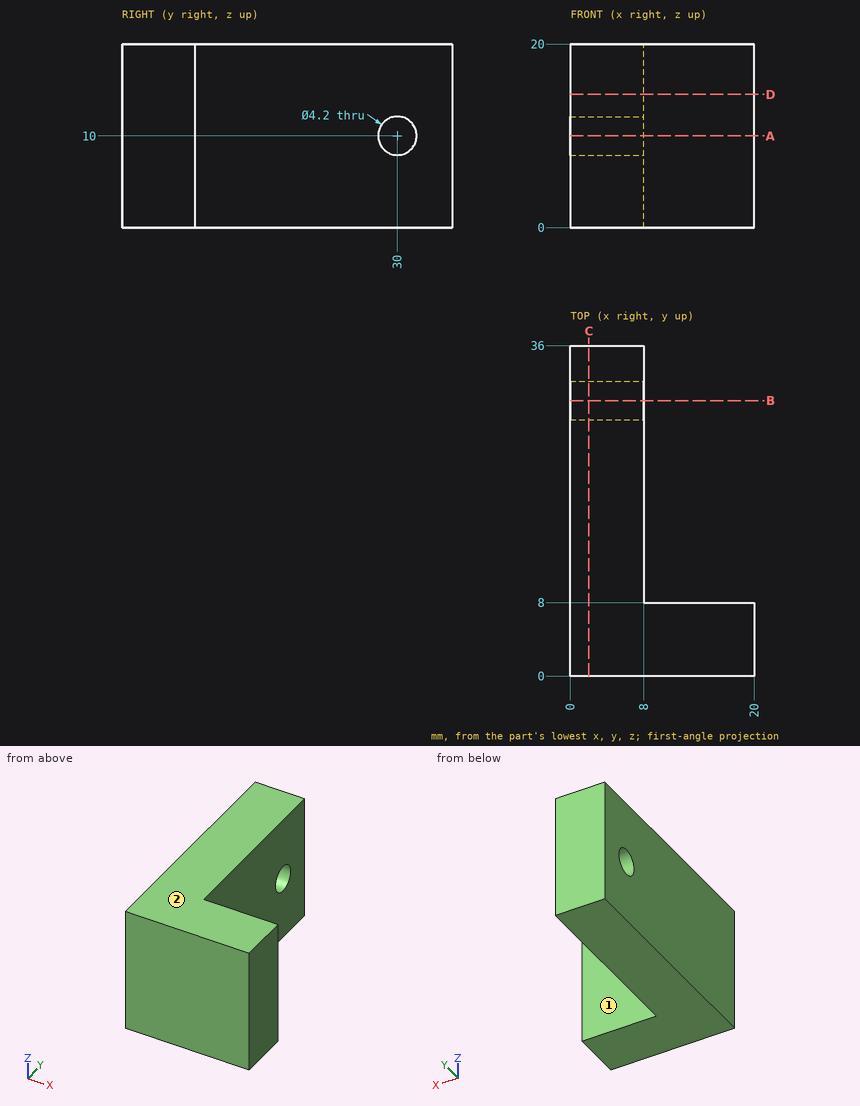
Could you check a few things on this drawing? It's one solid part, dimensions in mm from its lowest x, y, z. A direction names the side the tool comes from. Give positions to 0.01 mm unless a question says otherwise; leave off trailing zeros. Order: outer loops, then holes, each group sorted by start corner. A loop starts at its lowest first (then second) coordinate and runs counter-clockwise, first axis right, second up. Notation, with made-up numbers: (64, 61.5) - (106, 61.5) arc R20 ccw to (106, 78.5) - close; hole circle Ø11 at (21, 19.5). An arc over 180 degrees is marked (long way). Answer as a JSON object with one key per item and string values. Group by question number.
Item 1: Which directions (+Z, -Z, +X, -X, +Y, -Y) give clear straight access to the entire face, cutting with the end or side of a thin tool? Please do the marked faces 1 and 2.
Item 2: For P1, Ø5.5, axis at y = 30, z = 10, coming from the +X side; P2, Ø9.5, axis at x = 14, z = 8.5, coming from the +Y side, each with a flat end and sliding along its axis, tell me the tip position at first contact or that it passes through.
Item 3: If we section it at C-C on x = 2: Please give me the cut outline in (y, z).
Item 4: If we section it at B-B on y = 30: Please give me the cut outline in (x, z).
Item 5: If we section it at A-A on z = 10: Please give me the cut outline in (x, y), and give its area (3 significant figures).
Item 6: If we section it at D-D on z = 14.5: Please give me the cut outline in (x, y).
Item 7: Please list where these lines run through material, in increasing order: probe 1 along Y at (x, z) = (4.25, 10); probe 2 along Z at (x, y) = (4, 30); probe 3 along X at (y, z) = (11, 12.25).
Result set:
{
 "1": {"face 1": "+Z, -Z, +X, +Y", "face 2": "+Z, +X, -X, +Y, -Y"},
 "2": {"P1": "x = 8", "P2": "y = 8"},
 "3": {"outline": "(0, 0) - (36, 0) - (36, 20) - (0, 20) - close; hole circle Ø4.2 at (30, 10)"},
 "4": {"outline": "(0, 0) - (8, 0) - (8, 7.9) - (0, 7.9) - close; (0, 12.1) - (8, 12.1) - (8, 20) - (0, 20) - close"},
 "5": {"outline": "(0, 0) - (20, 0) - (20, 8) - (8, 8) - (8, 27.9) - (0, 27.9) - close; (0, 32.1) - (8, 32.1) - (8, 36) - (0, 36) - close", "area": "350 mm²"},
 "6": {"outline": "(0, 0) - (20, 0) - (20, 8) - (8, 8) - (8, 36) - (0, 36) - close"},
 "7": {"probe 1": "0 to 27.9, 32.1 to 36", "probe 2": "0 to 7.9, 12.1 to 20", "probe 3": "0 to 8"}
}
